from build123d import *

# Parameters (mm, degrees)
SKETCH_1_W                = 120
SKETCH_1_H                = 220
EXTRUDE_1_DEPTH           = 10
HOLE_WIZARD_M6_1_D        = 5
HOLE_WIZARD_1_D           = 6.6
HOLE_WIZARD_1_CBORE_D     = 11
HOLE_WIZARD_1_CBORE_DEPTH = 6.8
CUT_EXTRUDE_1_REACH       = 127.698
SKETCH_6_R                = 30
HOLE_WIZARD_2_D           = 5.5
HOLE_WIZARD_2_CBORE_D     = 9.5
HOLE_WIZARD_2_CBORE_DEPTH = 5.7
HOLE_WIZARD_3_D           = 6.6
HOLE_WIZARD_3_CBORE_D     = 11
HOLE_WIZARD_3_CBORE_DEPTH = 6.8
HOLE_WIZARD_4_D           = 5.5
HOLE_WIZARD_4_CBORE_D     = 10
HOLE_WIZARD_4_CBORE_DEPTH = 5.7
FILLET_1_R                = 5


with BuildPart() as part:
    # 草图1 → 凸台-拉伸1 (new body)
    with BuildSketch(Plane.XY):
        Rectangle(SKETCH_1_W, SKETCH_1_H)
    extrude(amount=EXTRUDE_1_DEPTH)

    # M6 螺纹孔1 (through all)
    with Locations(Plane(origin=(0, 0, 0), x_dir=(-1, 0, 0), z_dir=(0, 0, -1))):
        with Locations((-40, 90), (-40, 50), (40, 90), (40, 50)):
            Hole(HOLE_WIZARD_M6_1_D / 2)

    # 打孔尺寸(%根据)内六角圆柱头螺钉的类型1 (through all)
    with Locations(Plane(origin=(0, 0, 0), x_dir=(-1, 0, 0), z_dir=(0, 0, -1))):
        with Locations((32, -75), (-18, -75), (32, 75), (-18, 75)):
            CounterBoreHole(HOLE_WIZARD_1_D / 2, HOLE_WIZARD_1_CBORE_D / 2, HOLE_WIZARD_1_CBORE_DEPTH)

    # 草图6 → 切除-拉伸1 (cut, up to next)
    with BuildSketch(Plane(origin=(0, 0, 0), x_dir=(-1, 0, 0), z_dir=(0, 0, -1)), mode=Mode.PRIVATE) as cut_extrude_1_sk1:
        Circle(SKETCH_6_R)
    cut_extrude_1_tool1 = extrude(cut_extrude_1_sk1.sketch, amount=-CUT_EXTRUDE_1_REACH, mode=Mode.PRIVATE) & part.part
    add(cut_extrude_1_tool1.solids().sort_by_distance((0, 0, 0))[0], mode=Mode.SUBTRACT)

    # 打孔尺寸(%根据)内六角圆柱头螺钉的类型2 (through all)
    with Locations(Plane.XY.offset(10)):
        with Locations((-55, -30), (-55, -90)):
            CounterBoreHole(HOLE_WIZARD_2_D / 2, HOLE_WIZARD_2_CBORE_D / 2, HOLE_WIZARD_2_CBORE_DEPTH)

    # 打孔尺寸(%根据)内六角圆柱头螺钉的类型3 (through all)
    with Locations(Plane.XY.offset(10)):
        with Locations((-20, -60), (30, -60)):
            CounterBoreHole(HOLE_WIZARD_3_D / 2, HOLE_WIZARD_3_CBORE_D / 2, HOLE_WIZARD_3_CBORE_DEPTH)

    # 打孔尺寸(%根据)内六角圆柱头螺钉的类型4 (through all)
    with Locations(Plane(origin=(0, 0, 0), x_dir=(-1, 0, 0), z_dir=(0, 0, -1))):
        with Locations((-54, 30), (-54, 90), (-54, -102)):
            CounterBoreHole(HOLE_WIZARD_4_D / 2, HOLE_WIZARD_4_CBORE_D / 2, HOLE_WIZARD_4_CBORE_DEPTH)

    # 圆角1
    fillet_1_edges = [part.edges().sort_by_distance(p)[0] for p in [
        (-60, 110, 5),
        (-60, -110, 5),
    ]]
    fillet(fillet_1_edges, radius=FILLET_1_R)


solid = part.part
Model file for the job. Use its own axes, mm. A direction names the side the tool comes from. Give positions to 0.01 mm unless a question says otherwise; leave off trailing zeros. Order: outer loops, then holes, each group sorted by start corner. A loop starts at its lowest first (then second) coordinate and runs counter-clockwise, first axis right, second up. Notation, with made-up numbers: M 31,-10.75 L 65,-10.75 A21 cw 65,4.25 Z; hole C 81.5,51.5 d7. An arc over 180 degrees is marked long. Put each result on its own line as item: value. Start each with the question number.
(1) Drill centre lines: L1, parallel to Y at x = -55, z = 1.7; L2, parallel to Y at x = 54, z = 4.5; L3, parallel to Y at x = 25.5, z = 9.75. Where is each one in solid material? Low to high. Write a range as [from, to].
(2) Pull direction Y, two halves, no side cores. Call faces 4 (the face through (-59, 108, 5)), 5 (the face through (-56.03, -94.637, 7.19)), 6 (the face through (-28, -23, 10)): released by +Y, released by -Y, zero draft, split by the parting line, or undercut.
(3) Band-saw the part on B-B on y = 50. Give the cut face in (x, z), then the cut area to 3 significant figures.
(4) Band-saw the part on C-C on x = 18. Give the cut face in (y, z).
(5) Tool access for faces 1 (the face through (51.8, -104.2, 5.7)), 2 (the face through (29.97, 1.32, 4.93)), 3 (the face through (-52, -30, 4.3)): list every direction of +Z, -Z, +X, -X, +Y, -Y with a clear straight run to the whole face (end or side of a thin tool).
(6) Band-saw the part on A-A on x = -40. Give the cut face in (y, z), then the cut area to 3 significant figures.
(7) Band-saw the part on D-D on y = 6.5. Give the cut face in (x, z).
(8) Pin check, flat tips, straight feed: pin 1 Ø12.5 at (x, y) = (-20, -60) entering from +Z; pin 2 Ø4.5 at (x, y) = (40, 90) entering from -Z; pin 3 Ø5.5 at (x, y) = (-34.5, 75) entering from -Z; pin 4 Ø6.5 at (x, y) = (54, 90) entering from -Z. Stop position of each tip, or through.
Results below:
1. L1: y = [-110, -92.75], [-87.25, -32.75], [-27.25, 110]
1. L2: y = [-110, -107], [-97, 25], [35, 85], [95, 110]
1. L3: y = [-110, -63.16], [-56.84, -15.8], [15.8, 110]
2. face 4: released by +Y
2. face 5: undercut
2. face 6: zero draft
3. outline: M -60,0 L -42.5,0 L -42.5,10 L -60,10 Z; M -37.5,0 L 37.5,0 L 37.5,10 L -37.5,10 Z; M 42.5,0 L 60,0 L 60,10 L 42.5,10 Z
3. area: 1,100 mm2
4. outline: M -110,0 L -80.5,0 L -80.5,6.8 L -78.3,6.8 L -78.3,10 L -110,10 Z; M -71.7,6.8 L -69.5,6.8 L -69.5,0 L -24,0 L -24,10 L -71.7,10 Z; M 24,0 L 69.5,0 L 69.5,6.8 L 71.7,6.8 L 71.7,10 L 24,10 Z; M 78.3,6.8 L 80.5,6.8 L 80.5,0 L 110,0 L 110,10 L 78.3,10 Z
5. face 1: -Z
5. face 2: +Z, -Z
5. face 3: +Z
6. outline: M -110,0 L 47.5,0 L 47.5,10 L -110,10 Z; M 52.5,0 L 87.5,0 L 87.5,10 L 52.5,10 Z; M 92.5,0 L 110,0 L 110,10 L 92.5,10 Z
6. area: 2,100 mm2
7. outline: M -60,0 L -29.29,0 L -29.29,10 L -60,10 Z; M 29.29,0 L 60,0 L 60,10 L 29.29,10 Z
8. pin 1: stops at z = 10
8. pin 2: passes through
8. pin 3: stops at z = 6.8
8. pin 4: stops at z = 5.7
